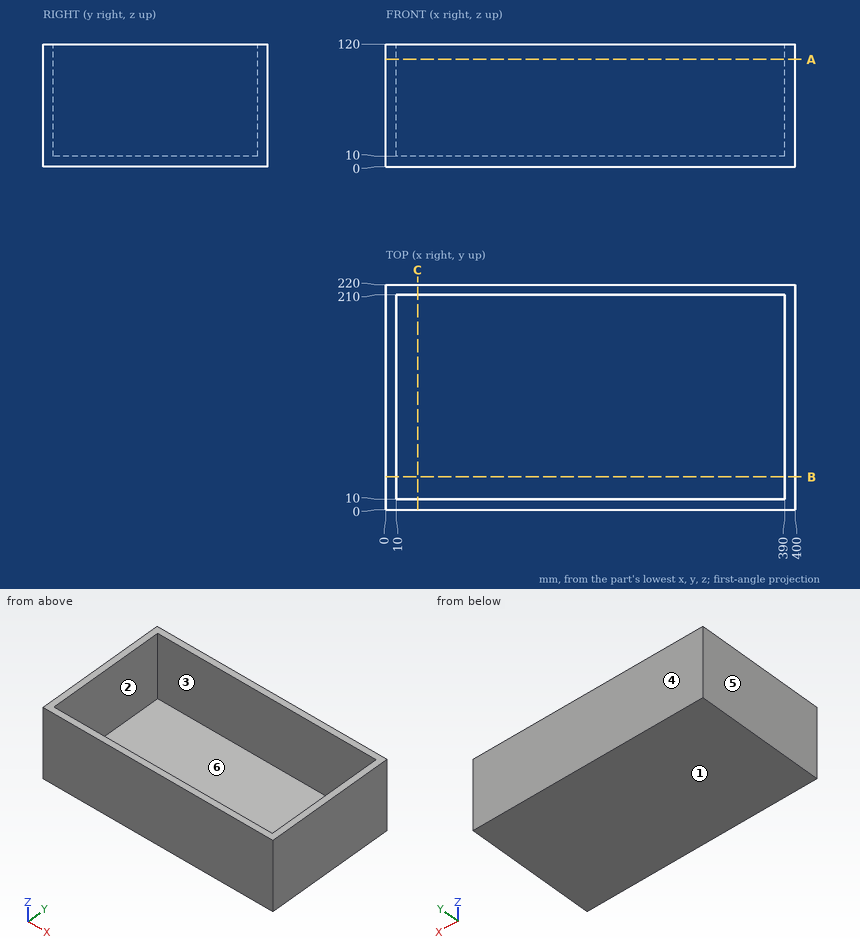
Part print with two shaded views. Sizes in mm from the minimum x, y, z corner. A direction names the side the tool comes from. Round coordinates to 2 decimals unless told otherwise and drop trailing zeros. Order: outer loops, then holes, each group sorted by start corner. A loop starts at its lowest first (then second) coordinate and runs counter-clockwise, first axis right, second up. Notation, with made-up numbers: M 57.5,-17.5 L 70.5,-17.5 A31 ccw 70.5,8.5 Z; hole C -31,-36 d5. An arc over 180 degrees is marked long. Put each result on its own line as item: value. Start each with the question number.
1. Two-plate mould, pull along Y, no slides. Class the marked faces 1, 2, 3 and 4: +Y half, -Y half, draft (parallel to the pull), parting line (faces both ways), or undercut.
2. Drop flat-ended pins along their axis: pin 1 (1 mm diameter, centred on y = 175, z = 72.5, fed in from -X); pin 2 (6 mm diameter, centred on x = 59.5, y = 90, fed in from +Z). Give the stop position or say it passes through.
3. Slice it at A-A on z = 105. List the corners of the cut face in (x, y).
4. Tool access for the marked faces 5 and 6: list every direction of +Z, -Z, +X, -X, +Y, -Y with a clear straight run to the whole face (end or side of a thin tool).
5. Slice it at B-B on y = 32. List the corners of the cut face in (x, z).
6. Slice it at C-C on x = 31. List the corners of the cut face in (y, z).
7. Drill centre lines: probe 1 along Y at (x, z) = (297.5, 17); probe 2 along X at (y, z) = (188, 69.5); probe 3 along Z at (x, y) = (244, 129). Where is each one in solid material? Low to high. Write a range as [from, to].
Findings:
1. face 1: draft
1. face 2: undercut
1. face 3: undercut
1. face 4: +Y half
2. pin 1: x = 0
2. pin 2: z = 10
3. outline: M 0,0 L 400,0 L 400,220 L 0,220 Z; hole M 10,10 L 390,10 L 390,210 L 10,210 Z
4. face 5: +Z, -Z, -X, +Y, -Y
4. face 6: +Z
5. outline: M 0,0 L 400,0 L 400,120 L 390,120 L 390,10 L 10,10 L 10,120 L 0,120 Z
6. outline: M 0,0 L 220,0 L 220,120 L 210,120 L 210,10 L 10,10 L 10,120 L 0,120 Z
7. probe 1: [0, 10], [210, 220]
7. probe 2: [0, 10], [390, 400]
7. probe 3: [0, 10]
